Work out the finished part from the listing and answer in its coordinate system (mm). A direction names the side the tool comes from. Give positions to 0.01 mm unless a question says otherwise; leave off trailing zeros. Put each result on its own line as item: value.
```python
from build123d import *

# Parameters (mm, degrees)
SKETCH_1_W                = 8
SKETCH_1_H                = 8
EXTRUDE_1_DEPTH           = 450
SKETCH_3_W                = 8
SKETCH_3_H                = 16
CUT_EXTRUDE_2_DEPTH       = 3
HOLE_WIZARD_M3_1_D        = 2.5
HOLE_WIZARD_M3_1_DEPTH    = 12
HOLE_WIZARD_M3_1_TIP      = 0.751075774
HOLE_WIZARD_M3_2_D        = 2.5
HOLE_WIZARD_M3_2_DEPTH    = 12
HOLE_WIZARD_M3_2_TIP      = 0.751075774
SKETCH_10_W               = 16
SKETCH_10_H               = 3
CUT_EXTRUDE_3_DEPTH       = 451.088880111
HOLE_WIZARD_1_D           = 3.4
HOLE_WIZARD_1_CBORE_D     = 6
HOLE_WIZARD_1_CBORE_DEPTH = 2


with BuildPart() as part:
    # 草图1 → 凸台-拉伸1 (new body)
    with BuildSketch(Plane.XY):
        Rectangle(SKETCH_1_W, SKETCH_1_H)
    extrude(amount=EXTRUDE_1_DEPTH)

    # 草图3 → 切除-拉伸2 (cut)
    with BuildSketch(Plane.XZ.offset(4)):
        with Locations((0, 420)):
            Rectangle(SKETCH_3_W, SKETCH_3_H)
    extrude(amount=-CUT_EXTRUDE_2_DEPTH, mode=Mode.SUBTRACT)

    # M3 螺纹孔1
    with Locations(Plane(origin=(0, 0, 0), x_dir=(-1, 0, 0), z_dir=(0, 0, -1))):
        with Locations((0, 0)):
            Hole(HOLE_WIZARD_M3_1_D / 2, depth=HOLE_WIZARD_M3_1_DEPTH)
            with Locations((0, 0, -(HOLE_WIZARD_M3_1_DEPTH + HOLE_WIZARD_M3_1_TIP / 2))):  # 118° drill point
                Cone(0, HOLE_WIZARD_M3_1_D / 2, HOLE_WIZARD_M3_1_TIP, mode=Mode.SUBTRACT)

    # M3 螺纹孔2
    with Locations(Plane.XY.offset(450)):
        with Locations((0, 0)):
            Hole(HOLE_WIZARD_M3_2_D / 2, depth=HOLE_WIZARD_M3_2_DEPTH)
            with Locations((0, 0, -(HOLE_WIZARD_M3_2_DEPTH + HOLE_WIZARD_M3_2_TIP / 2))):  # 118° drill point
                Cone(0, HOLE_WIZARD_M3_2_D / 2, HOLE_WIZARD_M3_2_TIP, mode=Mode.SUBTRACT)

    # 草图10 → 切除-拉伸3 (cut, through all)
    with BuildSketch(Plane(origin=(4, 0, 0), x_dir=(0, 0, -1), z_dir=(1, 0, 0))):
        with Locations((-320, -2.5)):
            Rectangle(SKETCH_10_W, SKETCH_10_H)
        with Locations((-220, -2.5)):
            Rectangle(SKETCH_10_W, SKETCH_10_H)
        with Locations((-120, -2.5)):
            Rectangle(SKETCH_10_W, SKETCH_10_H)
    extrude(amount=-CUT_EXTRUDE_3_DEPTH, mode=Mode.SUBTRACT)

    # 打孔尺寸根据内六角圆柱头螺钉的类型1 (through all)
    with Locations(Plane(origin=(0, 4, 0), x_dir=(1, 0, 0), z_dir=(0, 1, 0))):
        with Locations((0, -124), (0, -224), (0, -324), (0, -424)):
            CounterBoreHole(HOLE_WIZARD_1_D / 2, HOLE_WIZARD_1_CBORE_D / 2, HOLE_WIZARD_1_CBORE_DEPTH)


solid = part.part
```
(1) Straight lines are drawn through the part: line 1 (Z direction, x = 1.5, y = -1.5); line 2 (X direction, y = 1, z = 424); line 3 (Z direction, x = 0, y = -0.5). For each, find the intervals that lie inside material, in ascending order.
Geometry check:
line 1: z = 0 to 112, 128 to 212, 228 to 312, 328 to 412, 428 to 450
line 2: x = -4 to -1.7, 1.7 to 4
line 3: z = 12.45 to 122.3, 125.7 to 222.3, 225.7 to 322.3, 325.7 to 422.3, 425.7 to 437.55
(2) Given pin 1 (2.5 mm diameter, centred on x = 1.5, z = 418.5, fed in from -Y); pin 2 (2 mm diameter, centred on x = 0, y = 0, fed in from -Z); pin 3 (1 mm diameter, centred on x = -0.5, y = -0.5, fed in from +Z); pin 4 (2 mm diameter, centred on x = 0, z = 224, fed in from -Y), each flat-ended and moving along its own axis, determine where each tip first touches the part or whether it passes through.
Geometry check:
pin 1: stops at y = -1
pin 2: stops at z = 12.15
pin 3: stops at z = 437.97
pin 4: passes through
(3) A tool of negligible diameter and unlimited length cuts with its end or side. For faces 1 (the face through (-3, 4, 222)), 2 (the face through (0, -1, 420)), from which of +Z, -Z, +X, -X, +Y, -Y can it reach the whole face along a straight path? Write none if from no direction.
Geometry check:
face 1: +Z, -Z, +X, -X, +Y
face 2: +X, -X, -Y
(4) Determine the mould class of faces 3 (the face through (-1, 1, 0)), 4 (the face through (0, -1, 320)), 5 (the face through (-4, 1, 222)) for opening direction Z: pulls with the +Z half, pulls with the -Z half, needs draft (parallel to the pull), parting line crosses it, or undercut.
Geometry check:
face 3: pulls with the -Z half
face 4: undercut
face 5: needs draft
